from build123d import *

# Parameters (mm, degrees)
BASE_PLATE_SKETCH_W                 = 200
BASE_PLATE_SKETCH_H                 = 110
BASE_PLATE_DEPTH                    = 20
SIDE_BRACKET_SKETCH_R               = 17
SIDE_BRACKET_WITH_PIVOT_HOLES_DEPTH = 20
MOUNTING_FOOT_SKETCH_R              = 15
MOUNTING_FOOT_SKETCH_W              = 70
MOUNTING_FOOT_SKETCH_H              = 20
MOUNTING_FOOT_DEPTH                 = 20
TAPERED_LUG_SKETCH_R                = 15
TAPERED_PIVOT_LUG_DEPTH             = 20
BUSHING_BOSS_SKETCH_R               = 25
BUSHING_BOSS_SKETCH_R_2             = 15
BUSHING_BOSS_50_DEPTH               = 40
BUSHING_START                       = -40
BUSHING_BORE_SKETCH_R               = 15
BUSHING_BORE_30_DEPTH               = 40


with BuildPart() as part:
    # Base Plate Sketch → Base Plate (new body)
    with BuildSketch(Plane(origin=(0, 0, 0), x_dir=(1, 0, 0), z_dir=(0, 1, 0))):
        Rectangle(BASE_PLATE_SKETCH_W, BASE_PLATE_SKETCH_H)
    extrude(amount=BASE_PLATE_DEPTH)

    # Side Bracket Sketch → Side Bracket With Pivot Holes (add)
    with BuildSketch(Plane(origin=(0, 20, 0), x_dir=(1, 0, 0), z_dir=(0, 1, 0))):
        with BuildLine():
            Line((100, 55), (100, -12.5))
            Line((100, -12.5), (171.596768069, -12.5))
            ThreePointArc((171.596768069, -12.5), (187.275841171, -20.083612979), (191.064512046, -37.083333333))
            ThreePointArc((191.064512046, -37.083333333), (225.385865095, -85.982980748), (270, -46.25))
            Line((270, -46.25), (270, 88.75))
            ThreePointArc((270, 88.75), (225.385865095, 128.482980748), (191.064512046, 79.583333333))
            ThreePointArc((191.064512046, 79.583333333), (187.275841171, 62.583612979), (171.596768069, 55))
            Line((171.596768069, 55), (100, 55))
        make_face()
        with Locations(Location((230, 88.75, 0), (0, 0, 270))):
            Circle(SIDE_BRACKET_SKETCH_R, mode=Mode.SUBTRACT)
        with Locations(Location((230, -46.25, 0), (0, 0, 270))):
            Circle(SIDE_BRACKET_SKETCH_R, mode=Mode.SUBTRACT)
    extrude(amount=-SIDE_BRACKET_WITH_PIVOT_HOLES_DEPTH)

    # Mounting Foot Sketch → Mounting Foot (add)
    # profile 1 of 2: a face of its own
    with BuildSketch(Plane.ZY.offset(100)):
        with BuildLine():
            Line((25, 170), (-65, 170))
            ThreePointArc((-65, 170), (-95, 140), (-65, 110))
            Line((-65, 110), (-15, 110))
            Line((-15, 110), (-15, 20))
            Line((-15, 20), (55, 20))
            Line((55, 20), (55, 140))
            ThreePointArc((55, 140), (46.213203436, 161.213203436), (25, 170))
        make_face()
        with Locations((-65, 140)):
            Circle(MOUNTING_FOOT_SKETCH_R, mode=Mode.SUBTRACT)
        with Locations((25, 140)):
            Circle(MOUNTING_FOOT_SKETCH_R, mode=Mode.SUBTRACT)
    # profile 2 of 2: a face of its own
    with BuildSketch(Plane.ZY.offset(100)):
        with Locations((20, 10)):
            Rectangle(MOUNTING_FOOT_SKETCH_W, MOUNTING_FOOT_SKETCH_H)
    extrude(amount=-MOUNTING_FOOT_DEPTH)

    # Tapered Lug Sketch → Tapered Pivot Lug (add)
    with BuildSketch(Plane(origin=(100, 0, 0), x_dir=(0, 0, -1), z_dir=(1, 0, 0))):
        with BuildLine():
            Line((-55, 60), (-55, 20))
            Line((-55, 20), (-12.5, 20))
            Line((-12.5, 20), (55, 20))
            Line((55, 20), (55, 60))
            Line((55, 60), (64.734513274, 206.017699115))
            Line((64.734513274, 206.017699115), (65, 210))
            ThreePointArc((65, 210), (40.489921368, 239.493402031), (7.009282442, 220.794430535))
            Line((7.009282442, 220.794430535), (-55, 60))
        make_face()
        with Locations((35, 210)):
            Circle(TAPERED_LUG_SKETCH_R, mode=Mode.SUBTRACT)
    extrude(amount=-TAPERED_PIVOT_LUG_DEPTH)

    # Bushing Boss Sketch → Bushing Boss Ø50 (add)
    with BuildSketch(Plane(origin=(0, 20, 0), x_dir=(1, 0, 0), z_dir=(0, 1, 0))):
        with Locations(Location((10, 0, 0), (0, 0, 270))):
            Circle(BUSHING_BOSS_SKETCH_R)
        with Locations(Location((10, 0, 0), (0, 0, 270))):
            Circle(BUSHING_BOSS_SKETCH_R_2, mode=Mode.SUBTRACT)
    extrude(amount=BUSHING_BOSS_50_DEPTH)

    # Bushing Bore Sketch → Bushing Bore Ø30 (cut)
    with BuildSketch(Plane(origin=(0, 20, 0), x_dir=(1, 0, 0), z_dir=(0, 1, 0)).offset(BUSHING_START)):
        with Locations(Location((10, 0, 0), (0, 0, 270))):
            Circle(BUSHING_BORE_SKETCH_R)
    extrude(amount=BUSHING_BORE_30_DEPTH, mode=Mode.SUBTRACT)


solid = part.part
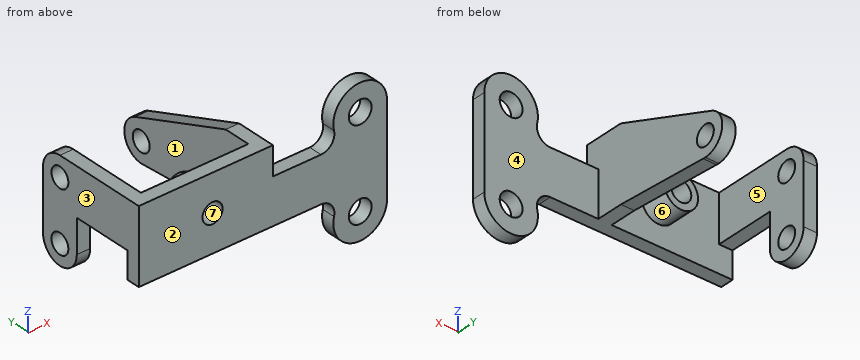
Model file for the job. Use its own axes, mm. Face numbers are marked on the shaded views. A direction names the side the tool comes from. Give positions to 0.01 mm unless a question says otherwise; leave off trailing zeros. Loops run counter-clockwise (first coordinate to the right, second up) from the corner with the lowest first, then second, coordinate; pieces in that order, holes last. Notation, with made-up numbers: (82, -21.75) -> (132, -21.75) arc R20 cw to (132, -3.75) -> close; hole circle Ø8 at (53, 42). An arc over 180 degrees is marked (long way). Use a Markdown table: item, result. Add a question column.
(1) Slice it at D-D on y = 131.5. List the corners of the cut face in (x, z).
(2) Tool access for the marked faces 4, 5, 6 and 7: list every direction of +Z, -Z, +X, -X, +Y, -Y with a clear straight run to the whole face (end or side of a thin tool).
(3) Wall check: line 1 along X through (y, z) = (48, 0); line 2 along Y through (x, z) = (-95.25, -65); line 3 along X through (y, z) = (99, 39). Give the ranges that are in metal, low to high.
(4) Slice it at B-B on z = 0. List the corners of the cut face in (x, y).
(5) Slice it at A-A on x = 10. List the corners of the cut face in (y, z), and give its area (3 significant figures).
(6) Mould opens along X. For the marked faces 1, 2 and 3 say: +X half, -X half, draft (parallel to the pull), parting line (faces both ways), or undercut.
(7) Slice it at C-C on y = 163.5. List the corners of the cut face in (x, z), and give its area (3 significant figures).
(8) Drop flat-ended pins along their axis: pin 1 Ø6 at (x, y) = (-85, 65.5) entering from -Z; pin 2 Ø10 at (x, y) = (127.5, 13.5) entering from +Z; pin 3 Ø6 at (x, z) = (-85.5, -15) entering from +Y. Give the stop position or say it passes through.
Filled sheet:
| question | item | result |
|---|---|---|
| 1 | outline | (-100, -93.77) -> (-80, -93.77) -> (-80, -77.36) -> (-100, -77.36) -> close; (-100, -52.64) -> (-80, -52.64) -> (-80, 12.64) -> (-100, 12.64) -> close; (-100, 37.36) -> (-80, 37.36) -> (-80, 55) -> (-100, 55) -> close; (80, -59.77) -> (100, -59.77) -> (100, 27.43) -> (80, 27.43) -> close |
| 2 | face 4 | +Z, -Z, +X, +Y |
| 2 | face 5 | +Z, -Z, +Y |
| 2 | face 6 | +Y |
| 2 | face 7 | +Y, -Y |
| 3 | line 1 | -100 to -80, -15 to -5, 25 to 35, 80 to 100 |
| 3 | line 2 | 110 to 125, 155 to 170 |
| 3 | line 3 | -100 to -80, 80 to 100 |
| 4 | outline | (-100, 0) -> (-5, 0) -> (-5, 60) -> (-15, 60) -> (-15, 20) -> (-80, 20) -> (-80, 170) -> (-100, 170) -> close; (25, 0) -> (270, 0) -> (270, 20) -> (100, 20) -> (100, 202.62) -> (80, 202.62) -> (80, 20) -> (35, 20) -> (35, 60) -> (25, 60) -> close |
| 5 | outline | (0, -55) -> (20, -55) -> (20, -25) -> (60, -25) -> (60, -15) -> (0, -15) -> close; (0, 15) -> (60, 15) -> (60, 25) -> (20, 25) -> (20, 55) -> (0, 55) -> close |
| 5 | area | 2,400 mm2 |
| 6 | face 1 | undercut |
| 6 | face 2 | draft |
| 6 | face 3 | -X half |
| 7 | outline | (-100, -83.65) -> (-80, -83.65) -> (-80, 43.65) -> (-100, 43.65) -> close; (80, -61.9) -> (100, -61.9) -> (100, 15.09) -> (80, 15.09) -> close |
| 7 | area | 4,090 mm2 |
| 8 | pin 1 | z = -15 |
| 8 | pin 2 | z = 12.5 |
| 8 | pin 3 | y = 170 |
